Model file for the job. Use its own axes, mm. Round coordinates to 2 decimals unless told otherwise and drop trailing zeros. Loops run counter-clockwise (first coordinate to the right, second up) from the corner with the lowest first, then second, coordinate; pieces in that order, holes last. Notation, with made-up numbers: M 56.25,5.25 L 74.25,5.25 A28 cw 74.25,39.25 Z; hole C 75.25,0.25 d7. An arc over 180 degrees is marked long. Use a Markdown table: item, result. Add a question column.
Item 1: Two-plate mould, pull along X, no slides. Class faces 1 (the flat face through (0, -13.5, 2)), 2 (the flat face through (9, 0, 2)), 3 (the cylindrical face through (-1.315, 4.496, 2.028)): +X half, -X half, draft (parallel to the pull), parting line (faces both ways), or undercut.
Item 2: Saw through at A-A on x = 3.75. Write the cut outline in (y, z).
Item 3: Wall check: L1, parallel to Y at x = 3.75, z = 1.4. Give the ranges that are in metal, low to high. Write a range as from..to.
Item 4: Saw through at C-C on z = 2.55. Give the number of separate pieces and of enclosed holes in the cut face, then the cut area to 3 significant figures.
Item 5: Saw through at B-B on y = 0. Write the cut outline in (x, z), then the cut area to 3 significant figures.
```python
from build123d import *

# Parameters (mm, degrees)
SKETCH_1_W               = 18
SKETCH_1_H               = 27
EXTRUDE_1_DEPTH          = 4
CUT_EXTRUDE_1_REACH      = 18.711
SKETCH_2_R               = 0.5
PATTERN_LINEAR_2_COUNT   = 3
PATTERN_LINEAR_2_PITCH   = 4
MIRROR_1_COPY_1_REACH    = 18.711
MIRROR_1_COPY_1_SKETCH_R = 0.5
MIRROR_1_COPY_2_REACH    = 18.711
MIRROR_1_COPY_2_SKETCH_R = 0.5


with BuildPart() as part:
    # Sketch 1 → Extrude 1 (new body)
    with BuildSketch(Plane.XY):
        Rectangle(SKETCH_1_W, SKETCH_1_H)
    extrude(amount=EXTRUDE_1_DEPTH)

    # Sketch 2 → Cut-Extrude 1 (cut, up to next)
    with BuildSketch(Plane.XY.offset(4), mode=Mode.PRIVATE) as cut_extrude_1_sk1:
        with Locations((-1.25, 0)):
            Circle(SKETCH_2_R)
    cut_extrude_1_tool1 = extrude(cut_extrude_1_sk1.sketch, amount=-CUT_EXTRUDE_1_REACH, mode=Mode.PRIVATE) & part.part
    # Sketch 2 → Cut-Extrude 1 (cut, up to next)
    with BuildSketch(Plane.XY.offset(4), mode=Mode.PRIVATE) as cut_extrude_1_sk2:
        with Locations((-3.75, 0)):
            Circle(SKETCH_2_R)
    cut_extrude_1_tool2 = extrude(cut_extrude_1_sk2.sketch, amount=-CUT_EXTRUDE_1_REACH, mode=Mode.PRIVATE) & part.part
    # Sketch 2 → Cut-Extrude 1 (cut, up to next)
    with BuildSketch(Plane.XY.offset(4), mode=Mode.PRIVATE) as cut_extrude_1_sk3:
        with Locations((1.25, 0)):
            Circle(SKETCH_2_R)
    cut_extrude_1_tool3 = extrude(cut_extrude_1_sk3.sketch, amount=-CUT_EXTRUDE_1_REACH, mode=Mode.PRIVATE) & part.part
    # Sketch 2 → Cut-Extrude 1 (cut, up to next)
    with BuildSketch(Plane.XY.offset(4), mode=Mode.PRIVATE) as cut_extrude_1_sk4:
        with Locations((3.75, 0)):
            Circle(SKETCH_2_R)
    cut_extrude_1_tool4 = extrude(cut_extrude_1_sk4.sketch, amount=-CUT_EXTRUDE_1_REACH, mode=Mode.PRIVATE) & part.part
    cut_extrude_1_1 = cut_extrude_1_tool1.solids().sort_by_distance((-1.25, 0, 4))[0]
    add(cut_extrude_1_1, mode=Mode.SUBTRACT)
    cut_extrude_1_2 = cut_extrude_1_tool2.solids().sort_by_distance((-3.75, 0, 4))[0]
    add(cut_extrude_1_2, mode=Mode.SUBTRACT)
    cut_extrude_1_3 = cut_extrude_1_tool3.solids().sort_by_distance((1.25, 0, 4))[0]
    add(cut_extrude_1_3, mode=Mode.SUBTRACT)
    cut_extrude_1_4 = cut_extrude_1_tool4.solids().sort_by_distance((3.75, 0, 4))[0]
    add(cut_extrude_1_4, mode=Mode.SUBTRACT)
    cut_extrude_1 = cut_extrude_1_1 + cut_extrude_1_2 + cut_extrude_1_3 + cut_extrude_1_4  # Cut-Extrude 1 as one shape, for the pattern or mirror that repeats it

    # Pattern Linear 2: Cut-Extrude 1 ×3
    with Locations(*[(0, -i * PATTERN_LINEAR_2_PITCH, 0) for i in range(1, PATTERN_LINEAR_2_COUNT)]):
        add(cut_extrude_1, mode=Mode.SUBTRACT)

    # Mirror 1 copy 1 sketch → Mirror 1 copy 1 (cut, up to next)
    with BuildSketch(Plane(origin=(0, 4, 4), x_dir=(1, 0, 0), z_dir=(0, 0, 1)), mode=Mode.PRIVATE) as mirror_1_copy_1_sk1:
        with Locations((-1.25, 0)):
            Circle(MIRROR_1_COPY_1_SKETCH_R)
    mirror_1_copy_1_tool1 = extrude(mirror_1_copy_1_sk1.sketch, amount=-MIRROR_1_COPY_1_REACH, mode=Mode.PRIVATE) & part.part
    # Mirror 1 copy 1 sketch → Mirror 1 copy 1 (cut, up to next)
    with BuildSketch(Plane(origin=(0, 4, 4), x_dir=(1, 0, 0), z_dir=(0, 0, 1)), mode=Mode.PRIVATE) as mirror_1_copy_1_sk2:
        with Locations((-3.75, 0)):
            Circle(MIRROR_1_COPY_1_SKETCH_R)
    mirror_1_copy_1_tool2 = extrude(mirror_1_copy_1_sk2.sketch, amount=-MIRROR_1_COPY_1_REACH, mode=Mode.PRIVATE) & part.part
    # Mirror 1 copy 1 sketch → Mirror 1 copy 1 (cut, up to next)
    with BuildSketch(Plane(origin=(0, 4, 4), x_dir=(1, 0, 0), z_dir=(0, 0, 1)), mode=Mode.PRIVATE) as mirror_1_copy_1_sk3:
        with Locations((1.25, 0)):
            Circle(MIRROR_1_COPY_1_SKETCH_R)
    mirror_1_copy_1_tool3 = extrude(mirror_1_copy_1_sk3.sketch, amount=-MIRROR_1_COPY_1_REACH, mode=Mode.PRIVATE) & part.part
    # Mirror 1 copy 1 sketch → Mirror 1 copy 1 (cut, up to next)
    with BuildSketch(Plane(origin=(0, 4, 4), x_dir=(1, 0, 0), z_dir=(0, 0, 1)), mode=Mode.PRIVATE) as mirror_1_copy_1_sk4:
        with Locations((3.75, 0)):
            Circle(MIRROR_1_COPY_1_SKETCH_R)
    mirror_1_copy_1_tool4 = extrude(mirror_1_copy_1_sk4.sketch, amount=-MIRROR_1_COPY_1_REACH, mode=Mode.PRIVATE) & part.part
    add(mirror_1_copy_1_tool1.solids().sort_by_distance((-1.25, 4, 4))[0], mode=Mode.SUBTRACT)
    add(mirror_1_copy_1_tool2.solids().sort_by_distance((-3.75, 4, 4))[0], mode=Mode.SUBTRACT)
    add(mirror_1_copy_1_tool3.solids().sort_by_distance((1.25, 4, 4))[0], mode=Mode.SUBTRACT)
    add(mirror_1_copy_1_tool4.solids().sort_by_distance((3.75, 4, 4))[0], mode=Mode.SUBTRACT)

    # Mirror 1 copy 2 sketch → Mirror 1 copy 2 (cut, up to next)
    with BuildSketch(Plane(origin=(0, 8, 4), x_dir=(1, 0, 0), z_dir=(0, 0, 1)), mode=Mode.PRIVATE) as mirror_1_copy_2_sk1:
        with Locations((-1.25, 0)):
            Circle(MIRROR_1_COPY_2_SKETCH_R)
    mirror_1_copy_2_tool1 = extrude(mirror_1_copy_2_sk1.sketch, amount=-MIRROR_1_COPY_2_REACH, mode=Mode.PRIVATE) & part.part
    # Mirror 1 copy 2 sketch → Mirror 1 copy 2 (cut, up to next)
    with BuildSketch(Plane(origin=(0, 8, 4), x_dir=(1, 0, 0), z_dir=(0, 0, 1)), mode=Mode.PRIVATE) as mirror_1_copy_2_sk2:
        with Locations((-3.75, 0)):
            Circle(MIRROR_1_COPY_2_SKETCH_R)
    mirror_1_copy_2_tool2 = extrude(mirror_1_copy_2_sk2.sketch, amount=-MIRROR_1_COPY_2_REACH, mode=Mode.PRIVATE) & part.part
    # Mirror 1 copy 2 sketch → Mirror 1 copy 2 (cut, up to next)
    with BuildSketch(Plane(origin=(0, 8, 4), x_dir=(1, 0, 0), z_dir=(0, 0, 1)), mode=Mode.PRIVATE) as mirror_1_copy_2_sk3:
        with Locations((1.25, 0)):
            Circle(MIRROR_1_COPY_2_SKETCH_R)
    mirror_1_copy_2_tool3 = extrude(mirror_1_copy_2_sk3.sketch, amount=-MIRROR_1_COPY_2_REACH, mode=Mode.PRIVATE) & part.part
    # Mirror 1 copy 2 sketch → Mirror 1 copy 2 (cut, up to next)
    with BuildSketch(Plane(origin=(0, 8, 4), x_dir=(1, 0, 0), z_dir=(0, 0, 1)), mode=Mode.PRIVATE) as mirror_1_copy_2_sk4:
        with Locations((3.75, 0)):
            Circle(MIRROR_1_COPY_2_SKETCH_R)
    mirror_1_copy_2_tool4 = extrude(mirror_1_copy_2_sk4.sketch, amount=-MIRROR_1_COPY_2_REACH, mode=Mode.PRIVATE) & part.part
    add(mirror_1_copy_2_tool1.solids().sort_by_distance((-1.25, 8, 4))[0], mode=Mode.SUBTRACT)
    add(mirror_1_copy_2_tool2.solids().sort_by_distance((-3.75, 8, 4))[0], mode=Mode.SUBTRACT)
    add(mirror_1_copy_2_tool3.solids().sort_by_distance((1.25, 8, 4))[0], mode=Mode.SUBTRACT)
    add(mirror_1_copy_2_tool4.solids().sort_by_distance((3.75, 8, 4))[0], mode=Mode.SUBTRACT)


solid = part.part
```
Entries:
| question | item | result |
|---|---|---|
| 1 | face 1 | draft |
| 1 | face 2 | +X half |
| 1 | face 3 | undercut |
| 2 | outline | M -13.5,0 L -8.5,0 L -8.5,4 L -13.5,4 Z; M -7.5,0 L -4.5,0 L -4.5,4 L -7.5,4 Z; M -3.5,0 L -0.5,0 L -0.5,4 L -3.5,4 Z; M 0.5,0 L 3.5,0 L 3.5,4 L 0.5,4 Z; M 4.5,0 L 7.5,0 L 7.5,4 L 4.5,4 Z; M 8.5,0 L 13.5,0 L 13.5,4 L 8.5,4 Z |
| 3 | L1 | -13.5..-8.5, -7.5..-4.5, -3.5..-0.5, 0.5..3.5, 4.5..7.5, 8.5..13.5 |
| 4 | separate pieces | 1 |
| 4 | enclosed holes | 20 |
| 4 | area | 470 mm2 |
| 5 | outline | M -9,0 L -4.25,0 L -4.25,4 L -9,4 Z; M -3.25,0 L -1.75,0 L -1.75,4 L -3.25,4 Z; M -0.75,0 L 0.75,0 L 0.75,4 L -0.75,4 Z; M 1.75,0 L 3.25,0 L 3.25,4 L 1.75,4 Z; M 4.25,0 L 9,0 L 9,4 L 4.25,4 Z |
| 5 | area | 56.0 mm2 |
